Read the model definition and answer for the solid it produces. Units are mm, in the model's axes. Coordinates: 2 decimals unless noted, no trailing zeros. Loops run counter-clockwise (first coordinate to the right, second up) from the corner with the lowest first, then second, coordinate; pieces in that order, holes last.
from build123d import *

# Parameters (mm, degrees)
SKETCH_1_R          = 130
SKETCH_1_R_2        = 10
EXTRUDE_1_DEPTH     = 5
SKETCH_2_R          = 50
CUT_EXTRUDE_1_DEPTH = 10


with BuildPart() as part:
    # 草图1 → 凸台-拉伸1 (new, symmetric)
    with BuildSketch(Plane.XY):
        Circle(SKETCH_1_R)
        with Locations((0, 108)):
            Circle(SKETCH_1_R_2, mode=Mode.SUBTRACT)
        with Locations((76.367532368, 76.367532368)):
            Circle(SKETCH_1_R_2, mode=Mode.SUBTRACT)
        with Locations((108, 0)):
            Circle(SKETCH_1_R_2, mode=Mode.SUBTRACT)
        with Locations((76.367532368, -76.367532368)):
            Circle(SKETCH_1_R_2, mode=Mode.SUBTRACT)
        with Locations((0, -108)):
            Circle(SKETCH_1_R_2, mode=Mode.SUBTRACT)
        with Locations((-76.367532368, -76.367532368)):
            Circle(SKETCH_1_R_2, mode=Mode.SUBTRACT)
        with Locations((-108, 0)):
            Circle(SKETCH_1_R_2, mode=Mode.SUBTRACT)
        with Locations((-76.367532368, 76.367532368)):
            Circle(SKETCH_1_R_2, mode=Mode.SUBTRACT)
    extrude(amount=EXTRUDE_1_DEPTH, both=True)

    # 草图2 → 切除-拉伸1 (cut)
    with BuildSketch(Plane.XY.offset(5)):
        Circle(SKETCH_2_R)
    extrude(amount=-CUT_EXTRUDE_1_DEPTH, mode=Mode.SUBTRACT)


solid = part.part
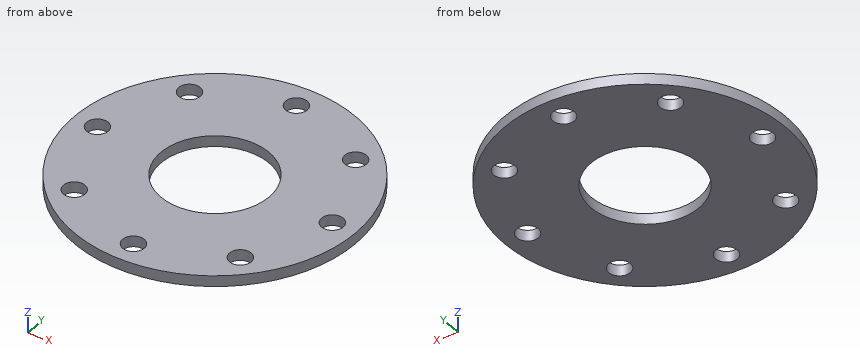
Item 1: A cutting plane is placed at B-B on y = 30. Determine the outline of the cut face in (x, z).
Numbers:
outline: (-126.49, -5) - (-40, -5) - (-40, 5) - (-126.49, 5) - close; (40, -5) - (126.49, -5) - (126.49, 5) - (40, 5) - close
Item 2: Given pin 1 (16 mm diameter, centred on x = -76.37, y = 76.37, fed in from +Z); pin 2 (1 mm diameter, centred on y = -27, z = -3.5, fed in from -X); pin 3 (4 mm diameter, centred on x = -69, z = -2, fed in from -Y); pin 4 (4 mm diameter, centred on x = 41.5, z = -2.5, fed in from -Y), each flat-ended and moving along its own axis, determine where each tip first touches the part or whether it passes through.
Numbers:
pin 1: passes through
pin 2: stops at x = -127.27
pin 3: stops at y = -111.4
pin 4: stops at y = -123.85
Item 3: Find the intervals of material crossed by line 1 along Y through (x, z) = (0, 2.75); line 2 along X through (y, z) = (-2, -1); line 3 along Y through (x, z) = (68.5, 2), in increasing order.
Numbers:
line 1: y = -130 to -118, -98 to -50, 50 to 98, 118 to 130
line 2: x = -129.98 to -117.8, -98.2 to -49.96, 49.96 to 98.2, 117.8 to 129.98
line 3: y = -110.49 to -82.54, -70.19 to 70.19, 82.54 to 110.49
Item 4: A cutting plane is placed at A-A on x = 0. Determine the outline of the cut face in (y, z).
Numbers:
outline: (-130, -5) - (-118, -5) - (-118, 5) - (-130, 5) - close; (-98, -5) - (-50, -5) - (-50, 5) - (-98, 5) - close; (50, -5) - (98, -5) - (98, 5) - (50, 5) - close; (118, -5) - (130, -5) - (130, 5) - (118, 5) - close
Item 5: A cutting plane is placed at D-D on x = -34. Determine the outline of the cut face in (y, z), then the cut area to 3 significant figures.
Numbers:
outline: (-125.48, -5) - (-36.66, -5) - (-36.66, 5) - (-125.48, 5) - close; (36.66, -5) - (125.48, -5) - (125.48, 5) - (36.66, 5) - close
area: 1,780 mm2
Item 6: A cutting plane is placed at C-C on z = 3.25. Give the number of separate pieces and of enclosed holes in the cut face, then the cut area to 3 significant figures.
Numbers:
separate pieces: 1
enclosed holes: 9
area: 42,700 mm2
